Can you work these out from the drawing? Everything is in mm from the part's minimum corner. Coordinates: 2 decimals unless noted, no trailing zeros. Order: outer loops, then holes, each group sorted by start corner. A loop starts at its lowest first (then second) coordinate and runs counter-clockwise, first axis right, second up. Notation, with made-up numbers: (84, -34) -> (118, -34) arc R23 ccw to (118, -13) -> close; hole circle Ø10 at (86.5, -36). An arc over 180 degrees is marked (long way). Return JSON: item names as keys, results as strings. Group by question number.
1) For pin 1 (1.5 mm diameter, centred on y = 18, z = 9, fed in from +X); pin 2 (3.5 mm diameter, centred on y = 8, z = 5, fed in from -X); pin 3 (5 mm diameter, centred on x = 17.5, z = 3, fed in from -Y) (1 decimal), each with a flat end and sliding along its axis, tell me the tip position at first contact or that it passes through.
2) If we section it at C-C, the plane x = 8.25: Please give me the cut outline in (y, z), then the cut area to 3 significant figures.
3) If I drill on probe 1 along Y at (x, z) = (5.25, 5); probe 2 along Y at (x, z) = (5, 6.25); probe 3 along Z at (x, y) = (6.25, 28), over which ranges is the centre line in solid material (lowest first)? Write a range as from..to.
4) If we section it at B-B, the plane y = 23.5: Please give me the cut outline in (x, z), then the cut area to 3 significant figures.
5) If we section it at D-D, the plane x = 19.5: Please give me the cut outline in (y, z).
6) If we section it at A-A, the plane z = 1.75: Please give me the cut outline in (x, y).
7) Thinking about a two-plate mould opening in Z: for the marked faces 1, 2 and 3, which applies, +Z half, -Z half, draft (parallel to the pull), parting line (faces both ways), or undercut?
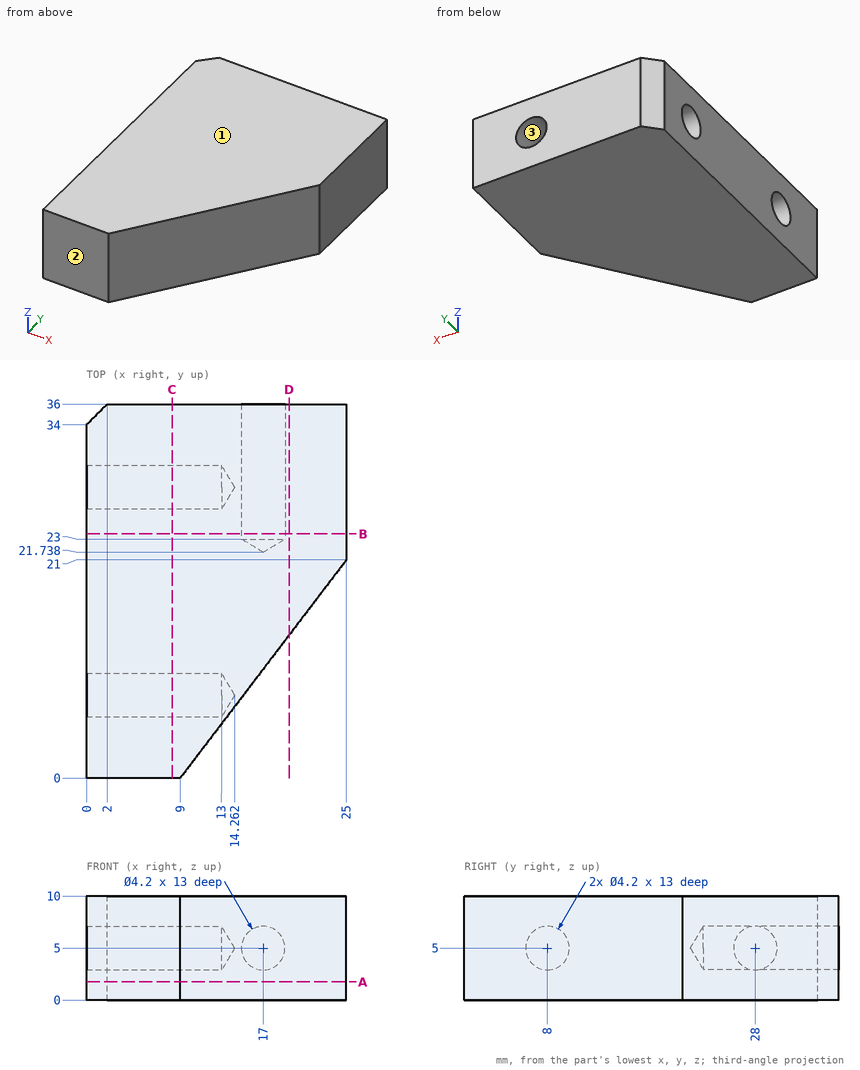
Result sheet:
{
 "1": {"pin 1": "stops at x = 23.29", "pin 2": "stops at x = 13.21", "pin 3": "stops at y = 7.9"},
 "2": {"outline": "(0, 0) -> (36, 0) -> (36, 10) -> (0, 10) -> close; hole circle Ø4.2 at (8, 5); hole circle Ø4.2 at (28, 5)", "area": "332 mm2"},
 "3": {"probe 1": "y = 0..5.9, 10.1..25.9, 30.1..36", "probe 2": "y = 0..6.31, 9.69..26.31, 29.69..36", "probe 3": "z = 0..2.9, 7.1..10"},
 "4": {"outline": "(0, 0) -> (25, 0) -> (25, 10) -> (0, 10) -> close; hole circle Ø4.2 at (17, 5)", "area": "236 mm2"},
 "5": {"outline": "(13.78, 0) -> (36, 0) -> (36, 10) -> (13.78, 10) -> close"},
 "6": {"outline": "(0, 0) -> (9, 0) -> (25, 21) -> (25, 36) -> (2, 36) -> (0, 34) -> close"},
 "7": {"face 1": "+Z half", "face 2": "draft", "face 3": "undercut"}
}
